Geometry check sheet. Reference: drawing and pictorial views, mm from the part's lowest x, y, z. A direction names the side the tool comes from. Give positions to 0.01 mm unless a question says otherwise; leave off trailing zeros. Order: outer loops, then holes, each group sorted by start corner. A loop starts at its lowest first (then second) coordinate and runs counter-clockwise, first axis right, second up. Notation, with made-up numbers: (-36.5, -16) - (-2.5, -16) arc R19 ccw to (-2.5, 17) - close; hole circle Ø7 at (3.5, 80.5). An arc over 180 degrees is marked (long way). Answer as a JSON object with one key per item and string values.
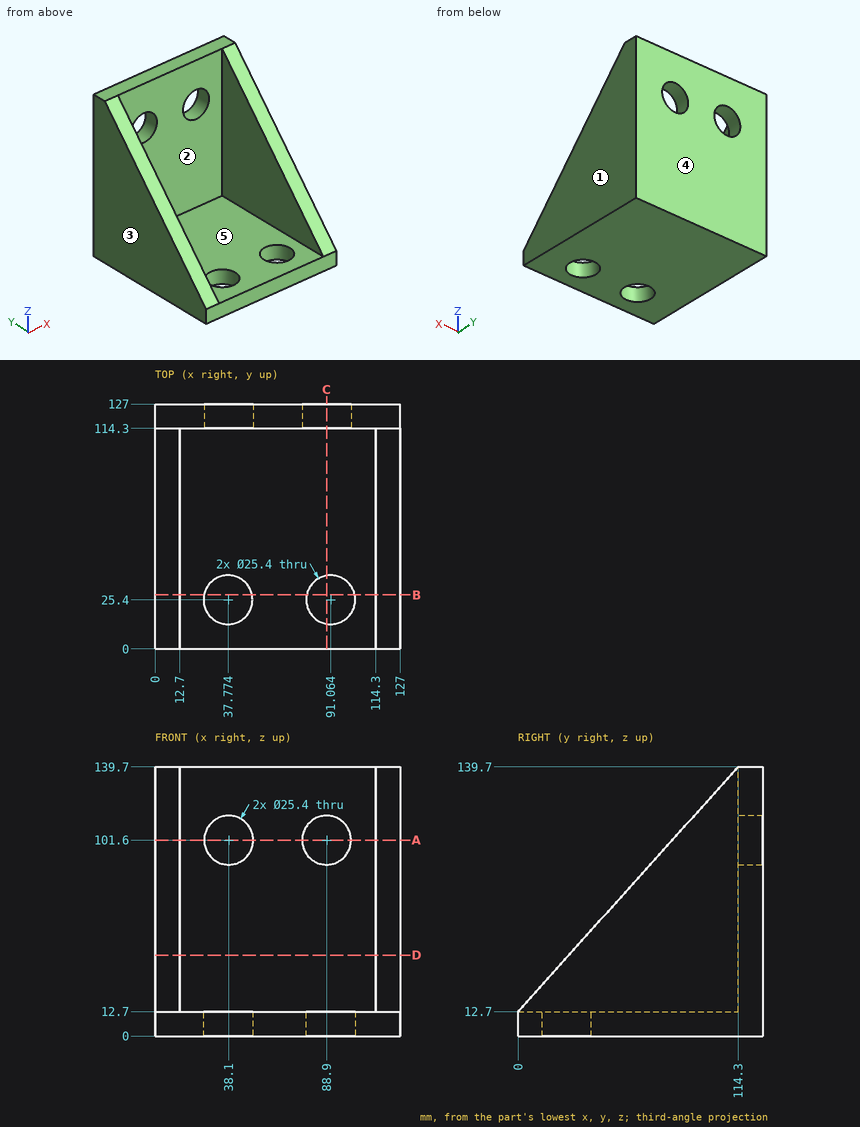
(1) Section check D-D (z = 42). Record the cut outline in (x, y), then the cut area to 3 significant figures.
Computed values:
{"outline": "(0, 26.37) - (12.7, 26.37) - (12.7, 114.3) - (114.3, 114.3) - (114.3, 26.37) - (127, 26.37) - (127, 127) - (0, 127) - close", "area": "3,850 mm²"}
(2) Material ranges on line 1 along X through (y, z) = (123.5, 101.6); line 2 along Z through (x, y) = (88, 124); line 3 along X through (y, z) = (106.5, 30.5), recorded low to high. Write a range as [from, to].
Computed values:
{"line 1": "x = [0, 25.4], [50.8, 76.2], [101.6, 127]", "line 2": "z = [0, 88.93], [114.27, 139.7]", "line 3": "x = [0, 12.7], [114.3, 127]"}
(3) Release check for a two-part mould opening along X. For the marked faces 3, 4 and 5 record: pulls with the +X half, pulls with the -X half, needs draft (parallel to the pull), parting line crosses it, or undercut.
Computed values:
{"face 3": "pulls with the -X half", "face 4": "needs draft", "face 5": "undercut"}
(4) Gauge pin test, flat end, axial feed: pin 1 Ø2 at (x, z) = (24, 42) entering from -Y. Record the tip position at first contact, or that the pin passes through.
Computed values:
{"pin 1": "stops at y = 114.3"}
(5) Section check C-C (x = 88.9). Record the cut outline in (y, z) (1 decimal).
Computed values:
{"outline": "(0, 0) - (12.9, 0) - (12.9, 12.7) - (0, 12.7) - close; (37.9, 0) - (127, 0) - (127, 88.9) - (114.3, 88.9) - (114.3, 12.7) - (37.9, 12.7) - close; (114.3, 114.3) - (127, 114.3) - (127, 139.7) - (114.3, 139.7) - close"}
(6) Section check B-B (y = 28). Record the cut outline in (x, z) (1 decimal).
Computed values:
{"outline": "(0, 0) - (25.3, 0) - (25.3, 12.7) - (12.7, 12.7) - (12.7, 43.8) - (0, 43.8) - close; (50.2, 0) - (78.6, 0) - (78.6, 12.7) - (50.2, 12.7) - close; (103.5, 0) - (127, 0) - (127, 43.8) - (114.3, 43.8) - (114.3, 12.7) - (103.5, 12.7) - close"}
(7) Access from +Z, -Z, +X, -X, +Y, -Y to the whole of each face (thin tool, end or side, straight path). Record for the marked faces 1 and 2.
Computed values:
{"face 1": "+Z, -Z, +X, +Y, -Y", "face 2": "+Z, -Y"}
(8) Section check A-A (z = 101.6). Record the cut outline in (x, y), then the cut area to 3 significant figures.
Computed values:
{"outline": "(0, 80.01) - (12.7, 80.01) - (12.7, 114.3) - (25.4, 114.3) - (25.4, 127) - (0, 127) - close; (50.8, 114.3) - (76.2, 114.3) - (76.2, 127) - (50.8, 127) - close; (101.6, 114.3) - (114.3, 114.3) - (114.3, 80.01) - (127, 80.01) - (127, 127) - (101.6, 127) - close", "area": "1,840 mm²"}
